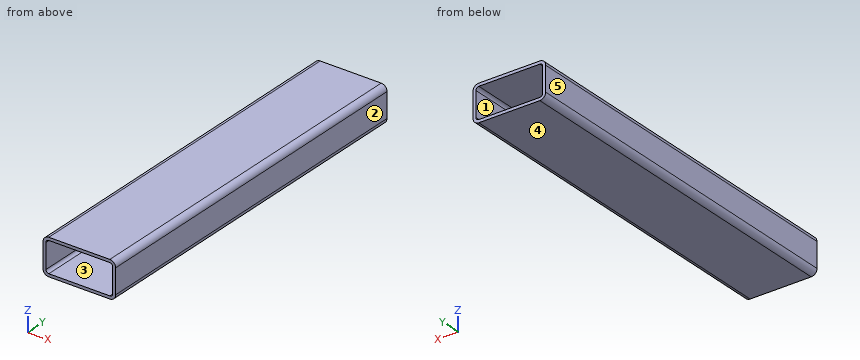
```python
from build123d import *

# Parameters (mm, degrees)
GB_T_6728_2002_RECTANGULAR_HOLLOW_SECTIO_DEPTH = 1000


with BuildPart() as part:
    # Sketch12 → GB/T 6728-2002 rectangular hollow section 200X100X8(2) (new body)
    with BuildSketch(Plane.ZX):
        with BuildLine():
            Line((-34, -100), (34, -100))
            ThreePointArc((34, -100), (45.313708499, -95.313708499), (50, -84))
            Line((50, -84), (50, 84))
            ThreePointArc((50, 84), (45.313708499, 95.313708499), (34, 100))
            Line((34, 100), (-34, 100))
            ThreePointArc((-34, 100), (-45.313708499, 95.313708499), (-50, 84))
            Line((-50, 84), (-50, -84))
            ThreePointArc((-50, -84), (-45.313708499, -95.313708499), (-34, -100))
        make_face()
        with BuildLine():
            Line((-34, -92), (34, -92))
            ThreePointArc((34, -92), (39.656854249, -89.656854249), (42, -84))
            Line((42, -84), (42, 84))
            ThreePointArc((42, 84), (39.656854249, 89.656854249), (34, 92))
            Line((34, 92), (-34, 92))
            ThreePointArc((-34, 92), (-39.656854249, 89.656854249), (-42, 84))
            Line((-42, 84), (-42, -84))
            ThreePointArc((-42, -84), (-39.656854249, -89.656854249), (-34, -92))
        make_face(mode=Mode.SUBTRACT)
    extrude(amount=GB_T_6728_2002_RECTANGULAR_HOLLOW_SECTIO_DEPTH)


solid = part.part
```
The listing builds one solid part. Answer for the finished solid, in the listing's coordinates (mm). Face numbers are marked on the shaded views. A direction names the side the tool comes from. Coordinates: 2 decimals unless noted, no trailing zeros. Write each loop counter-clockwise with the first axis right and the second up, starting at its lowest first coordinate (ties: lowest second). Pieces come first, ordered by that corner, then holes. Notation, with made-up numbers: (76.5, -14.75) - (99.5, -14.75) arc R9 ccw to (99.5, -2.75) - close; hole circle Ø8 at (55, 10). An arc over 180 degrees is marked (long way). Return JSON: item names as keys, results as strings. Group by question number.
Q1. Find the intervals of material crossed by line 1 along X through (y, z) = (667, 22); line 2 along Z through (x, y) = (61, 561); line 3 along X through (y, z) = (331, -35), in increasing order. Write a range as [from, to].
Q2. For a pull along Z with two mould halves and no side action, classify the marked faces 3, 4 and 5 as +Z half, -Z half, draft (parallel to the pull), parting line (faces both ways), or undercut.
Q3. The part is cut by section A-A on z = -21. Write down the section's boundary in (x, y), and give its area (3 significant figures).
Q4. The part is cut by section C-C on y = 505. Write down the section's boundary in (x, z).
Q5. The part is cut by section B-B on x = 50. Write down the section's boundary in (y, z), and give its area (3 significant figures).
Q6. Which of the six approach directions +Z, -Z, +X, -X, +Y, -Y give full straight-line access (tool end or side, diameter ignored) to the marked faces 1 and 2?
Q7. Flat-ended cylindrical pins translate along their axes: pin 1 Ø4 at (x, z) = (-0.5, -38.5) entering from +Y; pin 2 Ø1.5 at (y, z) = (456.5, 34.5) entering from +X. Find the tip coordinate at first contact, or state that the pin passes through.
Evaluation:
{
 "1": {"line 1": "x = [-100, -92], [92, 100]", "line 2": "z = [-50, -42], [42, 50]", "line 3": "x = [-99.97, -91.94], [91.94, 99.97]"},
 "2": {"face 3": "undercut", "face 4": "-Z half", "face 5": "draft"},
 "3": {"outline": "(-100, 0) - (-92, 0) - (-92, 1000) - (-100, 1000) - close; (92, 0) - (100, 0) - (100, 1000) - (92, 1000) - close", "area": "16,000 mm2"},
 "4": {"outline": "(-100, -34) arc R16 ccw to (-84, -50) - (84, -50) arc R16 ccw to (100, -34) - (100, 34) arc R16 ccw to (84, 50) - (-84, 50) arc R16 ccw to (-100, 34) - close; hole (-92, -34) arc R8 ccw to (-84, -42) - (84, -42) arc R8 ccw to (92, -34) - (92, 34) arc R8 ccw to (84, 42) - (-84, 42) arc R8 ccw to (-92, 34) - close"},
 "5": {"outline": "(0, -50) - (1000, -50) - (1000, -42) - (0, -42) - close; (0, 42) - (1000, 42) - (1000, 50) - (0, 50) - close", "area": "16,000 mm2"},
 "6": {"face 1": "+Y, -Y", "face 2": "+Z, -Z, +X, +Y, -Y"},
 "7": {"pin 1": "passes through", "pin 2": "stops at x = 100"}
}
